Build history of the part. All positions in model axes, mm. A direction names the side the tool comes from. Round coordinates to 2 decimals unless told otherwise and drop trailing zeros. Write each loop counter-clockwise with the first axis right and the second up, starting at its lowest first coordinate (ties: lowest second). Pieces come first, ordered by that corner, then holes.
Item 1: Drop flat-ended pins along their axis: pin 1 Ø24 at (x, z) = (10, 176) entering from -Y; pin 2 Ø5 at (y, z) = (572, 223.5) entering from -X; pin 3 Ø2 at (x, z) = (94.5, 122.5) entering from +Y. Give the stop position or say it passes through.
Item 2: Band-saw the part on B-B, the plane z = 349. Write the cut outline in (x, y), then the cut area to 3 significant figures.
Item 3: Band-saw the part on A-A, the plane y = 318.5. Write the cut outline in (x, z).
Item 4: 3-axis set-ups, long thin cutter, end or side, ignore diameter. For faces 4 (the flat face through (450, 349, 257)), 5 (the flat face through (0, 468, 222)), 6 (the flat face through (15, 168, 420)), 7 (the flat face through (177, 385, 450)): which of +Z, -Z, +X, -X, +Y, -Y reach the whole face in a straight line?
Item 5: Mould opens along X. For faces 1 (the flat face through (243, 370, 222)), 2 (the cylindrical face through (-3.343, 800.401, 221.85)), 3 (the flat face through (15, 0, 15)) say: +X half, -X half, draft (parallel to the pull), parting line (faces both ways), or undercut.
Item 6: Wall check: probe 1 along X at (y, z) = (63, 421); probe 2 along X at (y, z) = (615, 137.5); probe 3 along Y at (x, z) = (126.5, 204). Give the ranges that are in metal, low to high.
Item 7: Band-saw the part on C-C, the plane x = 232.5. Write the cut outline in (y, z).
Item 8: Band-saw the part on D-D, the plane y = 741. Write the cut outline in (x, z), then the cut area to 3 significant figures.
```python
from build123d import *

# Parameters (mm, degrees)
BOSS_EXTRUDE1_DEPTH = 450
SKETCH2_W           = 390
SKETCH2_H           = 365.797461664
CUT_EXTRUDE1_DEPTH  = 500


with BuildPart() as part:
    # Sketch1 → Boss-Extrude1 (new body)
    with BuildSketch(Plane.XY):
        with BuildLine():
            Line((0, 0), (0, 774.761772336))
            ThreePointArc((0, 774.761772336), (-3.437744681, 800.756595814), (-13.514616953, 824.964147969))
            Line((-13.514616953, 824.964147969), (-48.352023173, 884.979762437))
            ThreePointArc((-48.352023173, 884.979762437), (-48.369579018, 894.989870959), (-39.703484868, 900))
            Line((-39.703484868, 900), (-28.140837346, 900))
            ThreePointArc((-28.140837346, 900), (-23.150966388, 898.66609415), (-19.492299041, 895.020237563))
            Line((-19.492299041, 895.020237563), (12.430997961, 840.024860659))
            ThreePointArc((12.430997961, 840.024860659), (25.530931915, 808.555042857), (30, 774.761772336))
            Line((30, 774.761772336), (30, 400))
            Line((30, 400), (480, 400))
            Line((480, 400), (480, 0))
            Line((480, 0), (450, 0))
            Line((450, 0), (450, 370))
            Line((450, 370), (30, 370))
            Line((30, 370), (30, 0))
            Line((30, 0), (0, 0))
        make_face()
    extrude(amount=BOSS_EXTRUDE1_DEPTH)

    # Sketch2 → Cut-Extrude1 (cut)
    with BuildSketch(Plane(origin=(480, 0, 0), x_dir=(0, 0, -1), z_dir=(1, 0, 0))):
        with Locations((-225, 157.101269168)):
            Rectangle(SKETCH2_W, SKETCH2_H)
    extrude(amount=-CUT_EXTRUDE1_DEPTH, mode=Mode.SUBTRACT)


solid = part.part
```
Results:
1. pin 1: stops at y = 340
1. pin 2: stops at x = 0
1. pin 3: stops at y = 400
2. outline: (-48.35, 884.98) - (-13.51, 824.96) arc R100 cw to (0, 774.76) - (0, 340) - (30, 340) - (30, 370) - (450, 370) - (450, 340) - (480, 340) - (480, 400) - (30, 400) - (30, 774.76) arc R130 ccw to (12.43, 840.02) - (-19.49, 895.02) arc R10 ccw to (-28.14, 900) - (-39.7, 900) arc R10 ccw to start
2. area: 31,500 mm2
3. outline: (0, 0) - (30, 0) - (30, 30) - (0, 30) - close; (0, 420) - (30, 420) - (30, 450) - (0, 450) - close; (450, 0) - (480, 0) - (480, 30) - (450, 30) - close; (450, 420) - (480, 420) - (480, 450) - (450, 450) - close
4. face 4: +Z, -Z, -Y
4. face 5: +Z, -Z, -X, -Y
4. face 6: +X, -X, -Y
4. face 7: +Z, +X, -X, +Y, -Y
5. face 1: undercut
5. face 2: -X half
5. face 3: draft
6. probe 1: x = 0 to 30, 450 to 480
6. probe 2: x = 0 to 30
6. probe 3: y = 370 to 400
7. outline: (370, 0) - (400, 0) - (400, 450) - (370, 450) - close
8. outline: (0, 0) - (30, 0) - (30, 450) - (0, 450) - close
8. area: 13,500 mm2
